Check sheet for the modelled part. Datum: model origin and axes. Units: mm. Give positions to 0.01 mm unless a question says otherwise; leave off trailing zeros. Order: outer loops, then holes, each group sorted by start corner. A loop starts at its lowest first (then second) coordinate and runs counter-clockwise, first axis right, second up.
from build123d import *

# Parameters (mm, degrees)
SKETCH1_W           = 350
SKETCH1_H           = 100
BOSS_EXTRUDE1_DEPTH = 3
SKETCH2_W           = 3.2
SKETCH2_H           = 10.2
CUT_EXTRUDE1_DEPTH  = 183.027470454
SKETCH3_W           = 10
SKETCH3_H           = 3
BOSS_EXTRUDE2_DEPTH = 3


with BuildPart() as part:
    # Sketch1 → Boss-Extrude1 (new body)
    with BuildSketch(Plane(origin=(0, 0, 0), x_dir=(1, 0, 0), z_dir=(0, 1, 0))):
        Rectangle(SKETCH1_W, SKETCH1_H)
    extrude(amount=BOSS_EXTRUDE1_DEPTH)

    # Sketch2 → Cut-Extrude1 (cut, through all)
    with BuildSketch(Plane(origin=(0, 3, 0), x_dir=(1, 0, 0), z_dir=(0, 1, 0))):
        with Locations((-169, 25)):
            Rectangle(SKETCH2_W, SKETCH2_H)
        with Locations((-169, -30)):
            Rectangle(SKETCH2_W, SKETCH2_H)
        with Locations((169, -30)):
            Rectangle(SKETCH2_W, SKETCH2_H)
        with Locations((169, 25)):
            Rectangle(SKETCH2_W, SKETCH2_H)
    extrude(amount=-CUT_EXTRUDE1_DEPTH, mode=Mode.SUBTRACT)

    # Sketch3 → Boss-Extrude2 (add)
    with BuildSketch(Plane(origin=(0, 3, 0), x_dir=(1, 0, 0), z_dir=(0, 1, 0))):
        with Locations((-140, -51.5)):
            Rectangle(SKETCH3_W, SKETCH3_H)
        with Locations((0, -51.5)):
            Rectangle(SKETCH3_W, SKETCH3_H)
        with Locations((140, -51.5)):
            Rectangle(SKETCH3_W, SKETCH3_H)
    extrude(amount=-BOSS_EXTRUDE2_DEPTH)


solid = part.part
1) Section check C-C, the plane x = -20. Record the cut outline in (y, z).
Recorded:
outline: (0, -50) - (3, -50) - (3, 50) - (0, 50) - close
2) Section check B-B, the plane y = 2.15. State how many separate pieces and enclosed holes the cut face has, then the cut area to 3 significant figures.
Recorded:
separate pieces: 1
enclosed holes: 4
area: 35,000 mm2
3) Material ranges on L1, parallel to X at y = 1.8, z = 34.5; L2, parallel to Z at x = 103, y = 1.5, recorded low to high.
Recorded:
L1: x = -175 to -170.6, -167.4 to 167.4, 170.6 to 175
L2: z = -50 to 50
4) Depth check by flat-ended pin: pin 1 Ø0.9 at (x, y) = (-157.5, 1) entering from +Z; pin 2 Ø1.5 at (y, z) = (1, 51) entering from -X. Enter the tip coordinate at first touch or a pass-through.
Recorded:
pin 1: stops at z = 50
pin 2: stops at x = -145
5) Section check A-A, the plane z = 31. Record the cut outline in (x, y), then the cut area to 3 significant figures.
Recorded:
outline: (-175, 0) - (-170.6, 0) - (-170.6, 3) - (-175, 3) - close; (-167.4, 0) - (167.4, 0) - (167.4, 3) - (-167.4, 3) - close; (170.6, 0) - (175, 0) - (175, 3) - (170.6, 3) - close
area: 1,030 mm2
